```python
from build123d import *

# Parameters (mm, degrees)
SKETCH_1_W                  = 50
SKETCH_1_H                  = 34
EXTRUDE_1_DEPTH             = 6
HOLE_WIZARD_M5_1_AT_2_COUNT = 2
HOLE_WIZARD_M5_1_AT_2_PITCH = 35


with BuildPart() as part:
    # 草图1 → 凸台-拉伸1 (new, symmetric)
    with BuildSketch(Plane.XY):
        Rectangle(SKETCH_1_W, SKETCH_1_H)
    extrude(amount=EXTRUDE_1_DEPTH, both=True)

    # 草图3 → M5 螺纹孔1 (revolve, cut)
    with BuildSketch(Plane(origin=(-17.5, -17, 0), x_dir=(0, 0, -1), z_dir=(1, 0, 0))):
        Polygon((0, 0), (0, 13.6618073), (2.1, 12.4), (2.1, 0), align=None)
    hole_wizard_m5_1 = revolve(axis=Axis((-17.5, -23.35, 0), (0, 1, 0)), mode=Mode.SUBTRACT)

    # M5 螺纹孔1 at 2: M5 螺纹孔1 ×2
    with Locations(*[(i * HOLE_WIZARD_M5_1_AT_2_PITCH, 0, 0) for i in range(1, HOLE_WIZARD_M5_1_AT_2_COUNT)]):
        add(hole_wizard_m5_1, mode=Mode.SUBTRACT)

    # 镜向1: M5 螺纹孔1 across plane
    add(hole_wizard_m5_1.mirror(Plane.ZX), mode=Mode.SUBTRACT)

    # 镜向1 copy 1 sketch → 镜向1 copy 1 (revolve, cut)
    with BuildSketch(Plane(origin=(17.5, 17, 0), x_dir=(0, 0, -1), z_dir=(1, 0, 0))):
        Polygon((0, 0), (0, -13.6618073), (2.1, -12.4), (2.1, 0), align=None)
    revolve(axis=Axis((17.5, 23.35, 0), (0, 1, 0)), mode=Mode.SUBTRACT)


solid = part.part
```
The model under review builds one solid part; all positions refer to its coordinate system, in mm. A direction names the side the tool comes from. Give positions to 0.01 mm unless a question says otherwise; leave off trailing zeros. Write each loop counter-clockwise with the first axis right and the second up, starting at its lowest first coordinate (ties: lowest second). Pieces come first, ordered by that corner, then holes. Notation, with made-up numbers: (72.5, -6.5) - (106.5, -6.5) arc R27 ccw to (106.5, 10.5) - close; hole circle Ø11 at (76, 37.5). An arc over 180 degrees is marked (long way). Answer in a Markdown table with one row per item. Add a question column.
1. We need section A-A on y = -9. Write out the cut boundary in (x, z), then the cut area to 3 significant figures.
2. Tool access review of faces 4 (the cylindrical face through (15.418, 10.887, 0.273)), 5 (the flat face through (0, 0, -6)), 6 (the cylindrical face through (19.55, -10.89, 0.46)): name each direction out of +Z, -Z, +X, -X, +Y, -Y from which nothing blocks a thin tool from reaching the whole face with its end or side.
3. Draft analysis for pull direction X (two halves, no side actions). For faces 1 (the cylindrical face through (-19.27, -10.89, -1.13)), 2 (the flat face through (25, 0, 0)), 3 (the flat face through (0, -17, 0)), state which applies: +X half, -X half, draft (parallel to the pull), parting line (faces both ways), or undercut.
4. Wall thickness on line 1 along X through (y, z) = (9.25, 0); line 2 along X through (y, z) = (-13, -1.5); line 3 along Z through (x, y) = (17.5, 12): over which ranges is each line inside the solid? List them lowest first. Write a range as [from, to].
5. Insertion check: P1, Ø3.5, axis at x = 17.5, z = 0, coming from the +Y side; P2, Ø4, axis at x = 17.5, z = 0, coming from the +Y side; P3, Ø4, axis at x = -17.5, z = 0, coming from the -Y side. Each pin has a flat end and moves straight along its axis. Give the tip position at first contact, or say it passes through.
Ans:
| question | item | result |
|---|---|---|
| 1 | outline | (-25, -6) - (25, -6) - (25, 6) - (-25, 6) - close; hole circle Ø4.2 at (-17.5, 0); hole circle Ø4.2 at (17.5, 0) |
| 1 | area | 572 mm^2 |
| 2 | face 4 | +Y |
| 2 | face 5 | -Z, +X, -X, +Y, -Y |
| 2 | face 6 | -Y |
| 3 | face 1 | undercut |
| 3 | face 2 | +X half |
| 3 | face 3 | draft |
| 4 | line 1 | x = [-25, -19.6], [-15.4, 15.4], [19.6, 25] |
| 4 | line 2 | x = [-25, -18.97], [-16.03, 16.03], [18.97, 25] |
| 4 | line 3 | z = [-6, -2.1], [2.1, 6] |
| 5 | P1 | stops at y = 4.39 |
| 5 | P2 | stops at y = 4.54 |
| 5 | P3 | stops at y = -4.54 |
